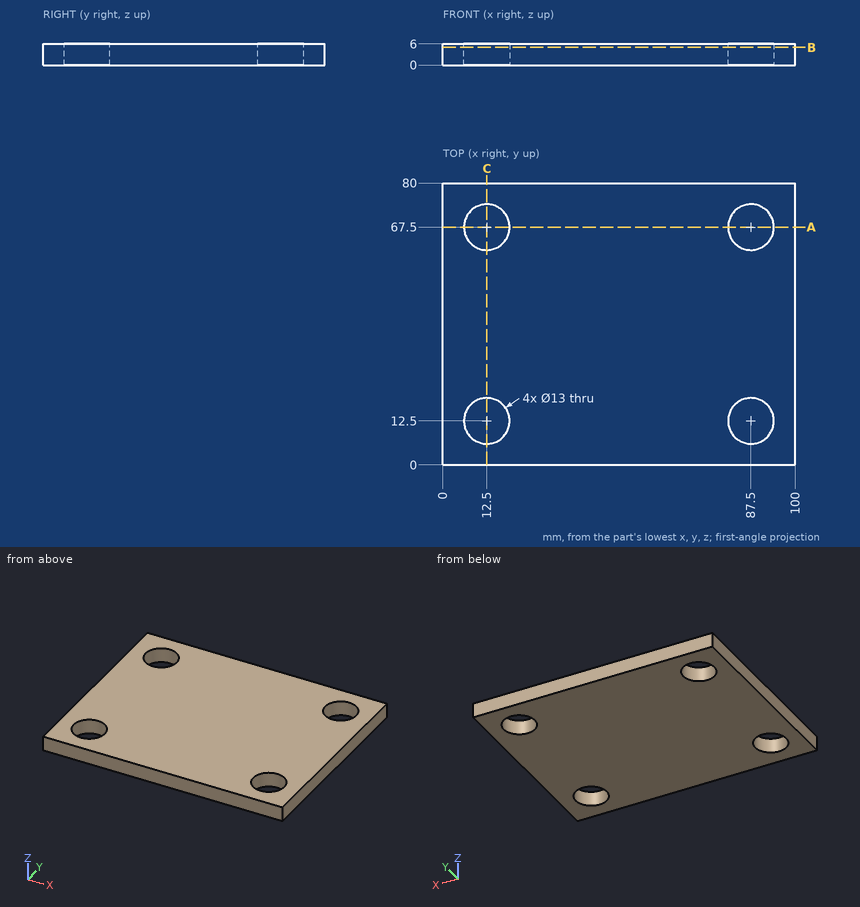
Can you work these out from the drawing? Everything is in mm from the part's minimum corner. Give positions to 0.01 mm unless a question says otherwise; leave off trailing zeros. Order: outer loops, then holes, each group sorted by start corner. A loop starts at its lowest first (then second) coordinate and runs counter-clockwise, first axis right, second up.
1. Will this pin go through, and if not, where does the flat tip stop? P1, Ø17, axis at x = 87.5, y = 67.5, coming from the +Z side.
2. Suppose I cut it at B-B (z = 5.05). List the corners of the cut face in (x, y) for me.
3. Suppose I cut it at A-A (y = 67.5). List the corners of the cut face in (x, z) for me.
4. Suppose I cut it at C-C (x = 12.5). List the corners of the cut face in (y, z) for me.
5. I need wall thicknesses on L1, parallel to Y at x = 12.5, z = 3.4; L2, parallel to Y at x = 18, z = 5.2; L3, parallel to X at y = 62.5, z = 5.3. Which ranges of each line are inside material? Lowest first, please.
Solved:
1. P1: stops at z = 6
2. outline: (0, 0) - (100, 0) - (100, 80) - (0, 80) - close; hole circle Ø13 at (12.5, 12.5); hole circle Ø13 at (12.5, 67.5); hole circle Ø13 at (87.5, 12.5); hole circle Ø13 at (87.5, 67.5)
3. outline: (0, 0) - (6, 0) - (6, 6) - (0, 6) - close; (19, 0) - (81, 0) - (81, 6) - (19, 6) - close; (94, 0) - (100, 0) - (100, 6) - (94, 6) - close
4. outline: (0, 0) - (6, 0) - (6, 6) - (0, 6) - close; (19, 0) - (61, 0) - (61, 6) - (19, 6) - close; (74, 0) - (80, 0) - (80, 6) - (74, 6) - close
5. L1: y = 0 to 6, 19 to 61, 74 to 80
5. L2: y = 0 to 9.04, 15.96 to 64.04, 70.96 to 80
5. L3: x = 0 to 8.35, 16.65 to 83.35, 91.65 to 100
